Verification items for the finished model (mm, model axes). A direction names the side the tool comes from. Coordinates: 2 decimals unless noted, no trailing zeros. Order: outer loops, then holes, each group sorted by start corner. A loop starts at its lowest first (then second) coordinate and runs counter-clockwise, first axis right, second up. Notation, with made-up numbers: M -33,5 L 10,5 A14 cw 10,28 Z; hole C 23,54.5 d4. An arc over 180 degrees is marked long. Write item = value, one per line.
```python
from build123d import *

# Parameters (mm, degrees)
CHAMFER_1_SIZE = 0.5


with BuildPart() as part:
    # 草图1 → 旋转1 (revolve)
    with BuildSketch(Plane(origin=(0, 0, 0), x_dir=(1, 0, 0), z_dir=(0, 1, 0)), mode=Mode.PRIVATE) as revolve_1_sk:
        Polygon((-28.614259258, 10.5), (13.385740742, 10.5), (13.385740742, 13), (21.385740742, 13), (21.385740742, 13.6), (22.685740742, 13.6), (22.685740742, 13), (24.385740742, 13), (24.385740742, 16), (-3.614259258, 16), (-3.614259258, 13), (-25.628618612, 13), (-28.614259258, 12.2), align=None)
    revolve(revolve_1_sk.sketch.rotate(Axis((0, 0, 0), (1, 0, 0)), 180), axis=Axis((0, 0, 0), (1, 0, 0)))

    # 倒角1
    chamfer_1_edges = [part.edges().sort_by_distance(p)[0] for p in [
        (-3.614259258, 0, -16),
        (24.385740742, 0, -13),
        (13.385740742, 0, -10.5),
        (-28.614259258, 0, -10.5),
    ]]
    chamfer(chamfer_1_edges, length=CHAMFER_1_SIZE)


solid = part.part
```
Item 1: Gauge pin test, flat ends, axial feed: pin 1 (1.5 mm diameter, centred on x = -10.5, y = 0.5, fed in from -Z); pin 2 (12.5 mm diameter, centred on y = 0, z = 0, fed in from -X); pin 3 (1 mm diameter, centred on x = -14.5, y = -5.5, fed in from -Z); pin 4 (6 mm diameter, centred on x = 6.5, y = 6.5, fed in from +Z). Record the tip position at first contact, or that the pin passes through.
Report:
pin_1 = -13
pin_2 = through
pin_3 = -12
pin_4 = 15.61
Item 2: Sectioned sample at D-D, the plane x = 18.5. Enter the section's corners in (y, z), then the cut area to 3 significant figures.
Report:
outline = C 0,0 d32; hole C 0,0 d26
area = 273 mm^2
Item 3: Sectioned sample at C-C, the plane x = -18.5. Enter the section's corners in (y, z), then the cut area to 3 significant figures.
Report:
outline = C 0,0 d26; hole C 0,0 d21
area = 185 mm^2
Item 4: Release check for a two-part mould opening along Y. For faces 1 (the conical face through (-28.469, -3.676, 11.674)), 2 (the flat face through (-28.614, -11, -2)), 3 (the flat face through (13.386, -3, 11)) record: pulls with the +Y half, pulls with the -Y half, needs draft (parallel to the pull), parting line crosses it, or undercut.
Report:
face_1 = parting line crosses it
face_2 = needs draft
face_3 = undercut
Item 5: Scan lines: L1, parallel to Y at x = 18.75, z = 0; L2, parallel to X at y = 9, z = -10; L3, parallel to X at y = -13.5, z = 5. Record each from-to range of solid material in increasing order. Write a range as from..to.
Report:
L1 = -16..-13, 13..16
L2 = -3.61..21.39, 22.69..24.34
L3 = -3.61..24.39
Item 6: Tool access check on faces 4 (the cylindrical face through (22.045, 13.277, -2.948)), 5 (the flat face through (-3.614, 13, 3)), 6 (the cylindrical face through (10.44, 15.62, -3.47)), 7 (the cylindrical face through (17.442, 7.91, -10.316)). Record the directions out of +Z, -Z, +X, -X, +Y, -Y that give a thin tool (end or side, any length) a straight path to the whole face; none if there is none.
Report:
face_4 = none
face_5 = -X
face_6 = +X, -X
face_7 = +X
